Design review of the part built by this model. Coordinates are the model's own, in mm. Give positions to 0.01 mm unless a question says otherwise; leave off trailing zeros. Write each loop counter-clockwise with the first axis right and the second up, starting at its lowest first coordinate (ties: lowest second). Pieces come first, ordered by that corner, then holes. Notation, with made-up numbers: (76.25, 57) -> (126.25, 57) arc R24 cw to (126.25, 75) -> close; hole circle Ø3 at (88.25, -3). An arc over 180 degrees is marked (long way). Use CSV: the item, a comma, the result in double quotes.
```python
from build123d import *

# Parameters (mm, degrees)
SKETCH1_W                  = 100
SKETCH1_H                  = 30
BOSS_EXTRUDE1_DEPTH        = 10
F_11_0_11_DIAMETER_HOLE1_D = 11


with BuildPart() as part:
    # Sketch1 → Boss-Extrude1 (new body)
    with BuildSketch(Plane(origin=(0, 0, 0), x_dir=(1, 0, 0), z_dir=(0, 1, 0))):
        Rectangle(SKETCH1_W, SKETCH1_H)
    extrude(amount=BOSS_EXTRUDE1_DEPTH)

    # Ø11.0 (11) Diameter Hole1 (through all)
    with Locations(Plane(origin=(0, 10, 0), x_dir=(1, 0, 0), z_dir=(0, 1, 0))):
        with Locations((-30, 0), (30, 0)):
            Hole(F_11_0_11_DIAMETER_HOLE1_D / 2)


solid = part.part
```
(1) For line 1 along Z through (x, y) = (-30, 5.5); line 2 along X through (y, z) = (4.25, 3.5); line 3 along Z through (x, y) = (34.5, 7), list the stretches that pass through material, from the lowest coordinate up. Write a range as [from, to].
Established:
line 1,"z = [-15, -5.5], [5.5, 15]"
line 2,"x = [-50, -34.24], [-25.76, 25.76], [34.24, 50]"
line 3,"z = [-15, -3.16], [3.16, 15]"
(2) Take a section at C-C (y = 8). Write out the cut boundary in (x, z), then the cut area to 3 significant figures.
Established:
outline,"(-50, -15) -> (50, -15) -> (50, 15) -> (-50, 15) -> close; hole circle Ø11 at (-30, 0); hole circle Ø11 at (30, 0)"
area,"2,810 mm2"
(3) Take a section at D-D (z = -3.75). Write out the cut boundary in (x, y).
Established:
outline,"(-50, 0) -> (-34.02, 0) -> (-34.02, 10) -> (-50, 10) -> close; (-25.98, 0) -> (25.98, 0) -> (25.98, 10) -> (-25.98, 10) -> close; (34.02, 0) -> (50, 0) -> (50, 10) -> (34.02, 10) -> close"
(4) Take a section at B-B (x = 30). Write out the cut boundary in (y, z), then the cut area to 3 significant figures.
Established:
outline,"(0, -15) -> (10, -15) -> (10, -5.5) -> (0, -5.5) -> close; (0, 5.5) -> (10, 5.5) -> (10, 15) -> (0, 15) -> close"
area,"190 mm2"
(5) Take a section at A-A (z = 0). Write out the cut boundary in (x, y), then the cut area to 3 significant figures.
Established:
outline,"(-50, 0) -> (-35.5, 0) -> (-35.5, 10) -> (-50, 10) -> close; (-24.5, 0) -> (24.5, 0) -> (24.5, 10) -> (-24.5, 10) -> close; (35.5, 0) -> (50, 0) -> (50, 10) -> (35.5, 10) -> close"
area,"780 mm2"
